Here's how the part is built. I have some questions about the finished solid (model axes, mm). Face numbers are marked on the shaded views. A direction names the side the tool comes from. Round coordinates to 2 decimals unless told otherwise and drop trailing zeros. Write each loop counter-clockwise with the first axis right and the second up, starting at its lowest first coordinate (ties: lowest second). Pieces come first, ordered by that corner, then holes. Notation, with made-up numbers: (45, -24) -> (87, -24) arc R30 cw to (87, 15) -> close; hole circle Ø4 at (20, 24.25). An arc over 180 degrees is marked (long way). Answer in a Markdown table with one row per item. Add a question column.
from build123d import *

# Parameters (mm, degrees)
BOSS_EXTRUDE1_DEPTH     = 5
CUT_EXTRUDE1_DEPTH      = 34.907195681
CUT_EXTRUDE1_DEPTH_BACK = 34.907195681
SKETCH2_R               = 2
SKETCH3_W               = 5.4
SKETCH3_H               = 10
CUT_EXTRUDE2_DEPTH      = 10
SKETCH4_R               = 2
CUT_EXTRUDE3_DEPTH      = 31
SKETCH7_W               = 5.4
SKETCH7_H               = 10
CUT_EXTRUDE5_DEPTH      = 13


with BuildPart() as part:
    # Sketch1 → Boss-Extrude1 (new, symmetric)
    with BuildSketch(Plane.XY):
        with BuildLine():
            Line((10.951340344, 4.304134495), (13.157250383, 20))
            ThreePointArc((13.157250383, 20), (18.804456232, 24.255474839), (23.059931071, 18.60826899))
            Line((23.059931071, 18.60826899), (20.854021031, 2.912403486))
            ThreePointArc((20.854021031, 2.912403486), (15.840885435, -6.320643703), (6, -10))
            Line((6, -10), (0, -10))
            ThreePointArc((0, -10), (-5, -5), (0, 0))
            Line((0, 0), (6, 0))
            ThreePointArc((6, 0), (9.280295145, 1.226452099), (10.951340344, 4.304134495))
        make_face()
    extrude(amount=BOSS_EXTRUDE1_DEPTH, both=True)

    # Sketch2 → Cut-Extrude1 (cut, two sides: drawn at the far end of the back side and taken through both)
    with BuildSketch(Plane.XY.offset(-CUT_EXTRUDE1_DEPTH_BACK)):
        with Locations((0, -5)):
            Circle(SKETCH2_R)
    extrude(amount=CUT_EXTRUDE1_DEPTH + CUT_EXTRUDE1_DEPTH_BACK, mode=Mode.SUBTRACT)

    # Sketch3 → Cut-Extrude2 (cut)
    with BuildSketch(Plane(origin=(-5, 0, 0), x_dir=(0, 0, -1), z_dir=(1, 0, 0))):
        with Locations((0, -5)):
            Rectangle(SKETCH3_W, SKETCH3_H)
    extrude(amount=CUT_EXTRUDE2_DEPTH, mode=Mode.SUBTRACT)

    # Sketch4 → Cut-Extrude3 (cut)
    with BuildSketch(Plane.XY.offset(5)):
        with Locations((18.108590727, 19.304134495)):
            Circle(SKETCH4_R)
    extrude(amount=-CUT_EXTRUDE3_DEPTH, mode=Mode.SUBTRACT)

    # Sketch7 → Cut-Extrude5 (cut)
    with BuildSketch(Plane(origin=(20.048712729, -2.817662822, 0), x_dir=(0, 0, -1), z_dir=(0.9902680687415704, -0.13917310096006613, 0))):
        with Locations((0, 21.636496711)):
            Rectangle(SKETCH7_W, SKETCH7_H)
    extrude(amount=-CUT_EXTRUDE5_DEPTH, mode=Mode.SUBTRACT)


solid = part.part
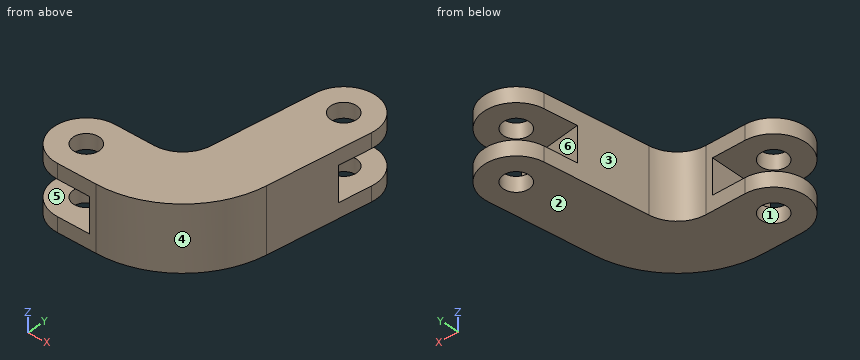
Item 1: On a 3-axis mill with a long thin cutter (end or side, diameter ignored), from which of +Z, -Z, +X, -X, +Y, -Y can I reach the whole of each face in a straight line? I mean the marked faces 4, 5 and 6. Say none if no direction works.
Item 2: If we section it at C-C on z = 1.5: Please give me the cut outline in (x, y).
Item 3: If we mould it in two halves opening along Y, with no side actions, what happens to the marked faces 1, 2 and 3? For each: pulls with the +Y half, pulls with the -Y half, needs draft (parallel to the pull), parting line crosses it, or undercut.
Item 4: I need wall thicknesses on line 1 along Z through (x, y) = (15.5, 18.5); line 2 along Y through (x, z) = (0, 3.9); line 3 along X through (y, z) = (-4, 4.25). Which ranges of each line are inside material? Lowest first, please. Write a range as from..to.
Item 5: If we section it at A-A on y = -6.5: Please give me the cut outline in (x, z).
Item 6: If we section it at D-D on x = 15.25: Please give me the cut outline in (y, z), then the cut area to 3 significant figures.
Item 7: For P1, Ø1.8, axis at x = 2.5, z = -2, coming from the +Y side; P2, Ø5, axis at x = 6.5, z = 0, coming from the -Y side; P3, Ø3.5, axis at x = 0, y = -5, coming from the +Z side; P4, Ø6, axis at y = -1, z = -3, coming from the +X side, each with a flat end and sliding along its axis, tell me the tip position at first contact or that it passes through.
Item 8: If we section it at B-B on z = -3.5: Please give me the cut outline in (x, y).
Results list:
| question | item | result |
|---|---|---|
| 1 | face 4 | +Z, -Z, +X, -Y |
| 1 | face 5 | -X, +Y, -Y |
| 1 | face 6 | +X, +Y |
| 2 | outline | (5, -10) -> (6, -10) arc R15 ccw to (20.85, 2.91) -> (22.36, 13.66) -> (12.46, 15.05) -> (10.95, 4.3) arc R5 cw to (6, 0) -> (5, 0) -> close |
| 3 | face 1 | undercut |
| 3 | face 2 | needs draft |
| 3 | face 3 | pulls with the +Y half |
| 4 | line 1 | -5..-2.7, 2.7..5 |
| 4 | line 2 | -10..-7, -3..0 |
| 4 | line 3 | -4.9..-1.73, 1.73..18 |
| 5 | outline | (-4.77, -5) -> (-1.32, -5) -> (-1.32, -2.7) -> (-4.77, -2.7) -> close; (-4.77, 2.7) -> (-1.32, 2.7) -> (-1.32, 5) -> (-4.77, 5) -> close; (1.32, -5) -> (15.63, -5) -> (15.63, 5) -> (1.32, 5) -> (1.32, 2.7) -> (5, 2.7) -> (5, -2.7) -> (1.32, -2.7) -> close |
| 6 | outline | (-6.81, -5) -> (23.41, -5) -> (23.41, -2.7) -> (14.66, -2.7) -> (14.66, 2.7) -> (23.41, 2.7) -> (23.41, 5) -> (-6.81, 5) -> close |
| 6 | area | 255 mm² |
| 7 | P1 | y = 0 |
| 7 | P2 | y = -10 |
| 7 | P3 | through |
| 7 | P4 | x = 20.7 |
| 8 | outline | (0, -10) -> (6, -10) arc R15 ccw to (20.85, 2.91) -> (23.06, 18.61) arc R5 ccw to (13.16, 20) -> (10.95, 4.3) arc R5 cw to (6, 0) -> (0, 0) arc R5 ccw to start; hole circle Ø4 at (0, -5); hole circle Ø4 at (18.11, 19.3) |
